The model under review builds one solid part; all positions refer to its coordinate system, in mm. Round coordinates to 2 decimals unless told otherwise and drop trailing zeros. Loops run counter-clockwise (first coordinate to the right, second up) from the corner with the lowest first, then second, coordinate; pieces in that order, holes last. Notation, with made-up numbers: (5, -30) -> (17, -30) arc R34 ccw to (17, 4) -> close; hole circle Ø4 at (-15.75, 51). An arc over 180 degrees is marked (long way). Write each question's results on one line, items separated by ' | '. Start each with the question number.
Item 1: We need section C-C (x = 24). Give the boundary of the cut face in (y, z).
Item 2: We need section D-D (y = -25). Give the boundary of the cut face in (x, z), and give its area (3 significant figures).
Item 3: We need section B-B (y = -14). Give the boundary of the cut face in (x, z), and give its area (3 significant figures).
Item 4: Clearance check with a flat-ended pin moving along its axis: pin 1 Ø2 at (x, z) = (23.5, 8) entering from -Y. State where the tip first meets the part, or that it passes through.
Item 5: For L1, parallel to Y at x = 16, z = 2; L2, parallel to Z at x = 25, y = 11; L3, parallel to Y at x = -26, z = 9, list the stretches that pass through material, from the lowest coordinate up. Write a range as from..to.
Item 6: We need section A-A (z = 4). Give the boundary of the cut face in (x, y), and give its area (3 significant figures).
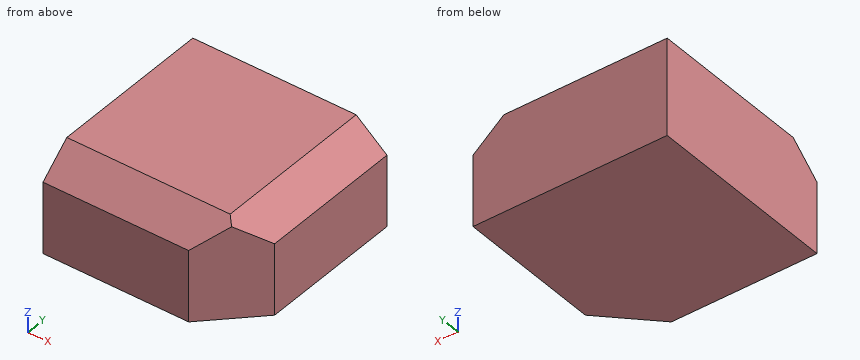
from build123d import *

# Parameters (mm, degrees)
SKETCH1_W           = 60
SKETCH1_H           = 60
BOSS_EXTRUDE1_DEPTH = 15
CHAMFER1_SIZE       = 15
CHAMFER2_SIZE       = 8
CHAMFER2_SIZE2      = 9.534028741
CHAMFER3_SIZE       = 8
CHAMFER3_SIZE2      = 9.534028741


with BuildPart() as part:
    # Sketch1 → Boss-Extrude1 (new, symmetric)
    with BuildSketch(Plane.XY):
        Rectangle(SKETCH1_W, SKETCH1_H)
    extrude(amount=BOSS_EXTRUDE1_DEPTH, both=True)

    # Chamfer1
    chamfer1_edges = [part.edges().sort_by_distance(p)[0] for p in [
        (30, -30, 0),
    ]]
    chamfer(chamfer1_edges, length=CHAMFER1_SIZE)

    # Chamfer2
    chamfer2_edges = [part.edges().sort_by_distance(p)[0] for p in [
        (-7.5, -30, 15),
    ]]
    chamfer2_side = [part.faces().sort_by_distance(p)[0] for p in [
        (-7.5, -30, 0),
    ]]
    chamfer(chamfer2_edges, length=CHAMFER2_SIZE, length2=CHAMFER2_SIZE2, reference=chamfer2_side[0])

    # Chamfer3
    chamfer3_edges = [part.edges().sort_by_distance(p)[0] for p in [
        (30, 7.5, 15),
    ]]
    chamfer3_side = [part.faces().sort_by_distance(p)[0] for p in [
        (30, 7.5, 0),
    ]]
    chamfer(chamfer3_edges, length=CHAMFER3_SIZE, length2=CHAMFER3_SIZE2, reference=chamfer3_side[0])


solid = part.part
Here are the results:
1) outline: (-21, -15) -> (30, -15) -> (30, 12.03) -> (-21, 12.03) -> close
2) outline: (-30, -15) -> (20, -15) -> (20, 11.2) -> (-30, 11.2) -> close | area: 1,310 mm2
3) outline: (-30, -15) -> (30, -15) -> (30, 7) -> (20.47, 15) -> (-30, 15) -> close | area: 1,760 mm2
4) pin 1: stops at y = -22.5
5) L1: y = -29..30 | L2: z = -15..11.2 | L3: y = -27.62..30
6) outline: (-30, -30) -> (15, -30) -> (30, -15) -> (30, 30) -> (-30, 30) -> close | area: 3,490 mm2
